Here's the drawing with two shaded views (mm, measured from the low corner). I have some questions. Round coordinates to 2 decimals unless told otherwise and drop trailing zeros. Order: outer loops, then holes, each group sorted by start corner. A loop starts at its lowest first (then second) coordinate and runs counter-clockwise, first axis right, second up.
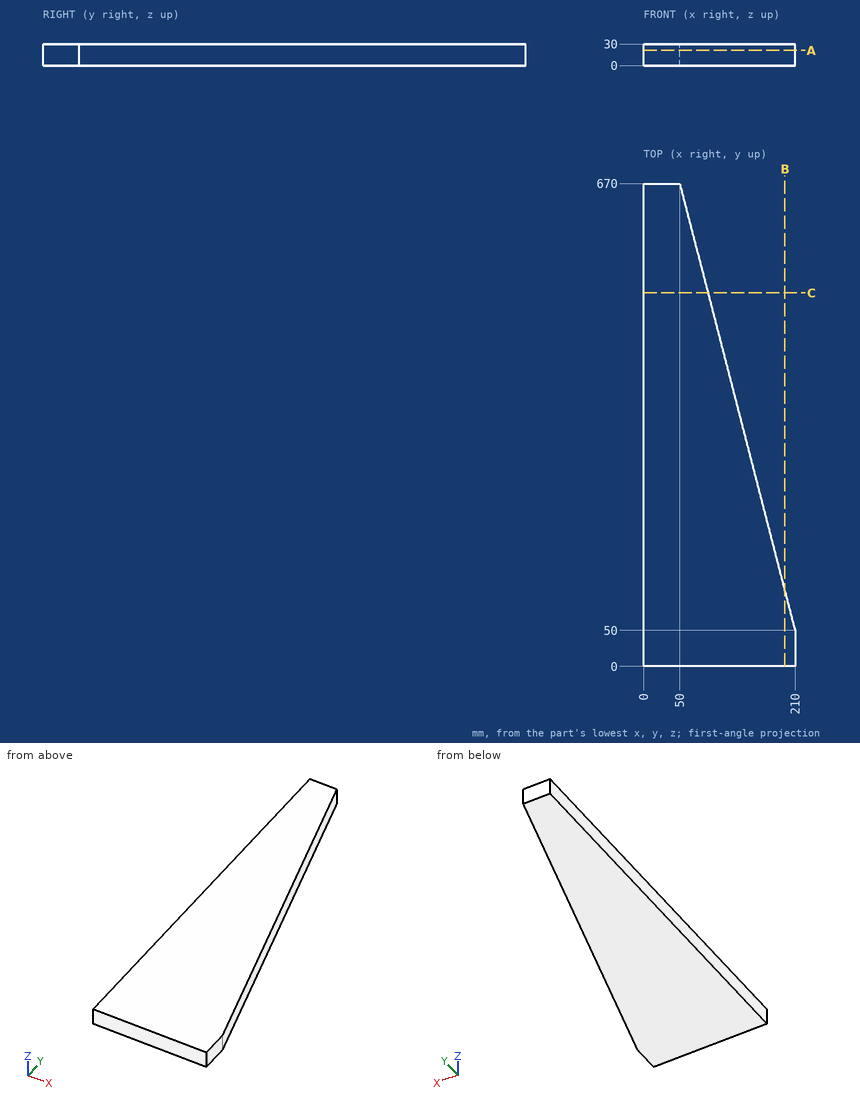
1. I'm going to push flat-ended pins straight in: P1, Ø12, axis at y = 419.5, z = 20.5, coming from the +X side; P2, Ø5, axis at y = 260.5, z = 13, coming from the +X side; P3, Ø6, axis at y = 403.5, z = 3.5, coming from the +X side. Where does each tip first touch, or does it pass through?
Evaluation:
P1: stops at x = 116.19
P2: stops at x = 156.32
P3: stops at x = 119.55
2. If we section it at A-A, the plane z = 21: Write out the boundary of the cut face in (x, y).
Evaluation:
outline: (0, 0) - (210, 0) - (210, 50) - (50, 670) - (0, 670) - close
3. I need wall thicknesses on probe 1 along X at (y, z) = (392.5, 4.5); probe 2 along X at (y, z) = (386.5, 27.5). Which ranges of each line are inside material? Lowest first, please.
Evaluation:
probe 1: x = 0 to 121.61
probe 2: x = 0 to 123.16
4. If we section it at C-C, the plane y = 518.5: Write out the boundary of the cut face in (x, z), and give its area (3 significant figures).
Evaluation:
outline: (0, 0) - (89.1, 0) - (89.1, 30) - (0, 30) - close
area: 2,670 mm2
5. If we section it at B-B, the plane x = 196: Write out the boundary of the cut face in (y, z), and give its area (3 significant figures).
Evaluation:
outline: (0, 0) - (104.25, 0) - (104.25, 30) - (0, 30) - close
area: 3,130 mm2
